Answer from the drawing. Dimensions are ordinates in mm from the lowest x, y and z of the part. Give positions to 0.01 mm unless a question says otherwise; leave off trailing zeros. Loops run counter-clockwise (first coordinate to the right, second up) from the corner with the lowest first, then second, coordinate; pieces in that order, holes last. Notation, with made-up numbers: (63.25, -17) -> (91.25, -17) arc R20 cw to (91.25, 15) -> close; hole circle Ø3 at (21.5, -24). An arc over 180 degrees is marked (long way). Write each question's results on one line, items separated by ' | '. Start each with the question number.
Item 1: Section A-A on z = 472 is taken. Write down the section's boundary in (x, y), and give its area (3 significant figures).
Item 2: Section B-B on x = 26.5 is taken. Write down the section's boundary in (y, z), and give its area (3 significant figures).
Item 3: Section C-C on y = 9 is taken. Write down the section's boundary in (x, z), and give its area (3 significant figures).
Item 4: Each of these flat-tipped pins is pushed along its axis until it touches: P1, Ø10, axis at x = 24, y = 36.5, coming from the -Z side; P2, Ø6, axis at x = 26, y = 35, coming from the +Z side. Where does it stop, or does it pass through?
Item 5: Find the intervals of material crossed by line 1 (X direction, y = 41.5, z = 467.5); line 2 (Z direction, x = 36.5, y = 62), in increasing order.
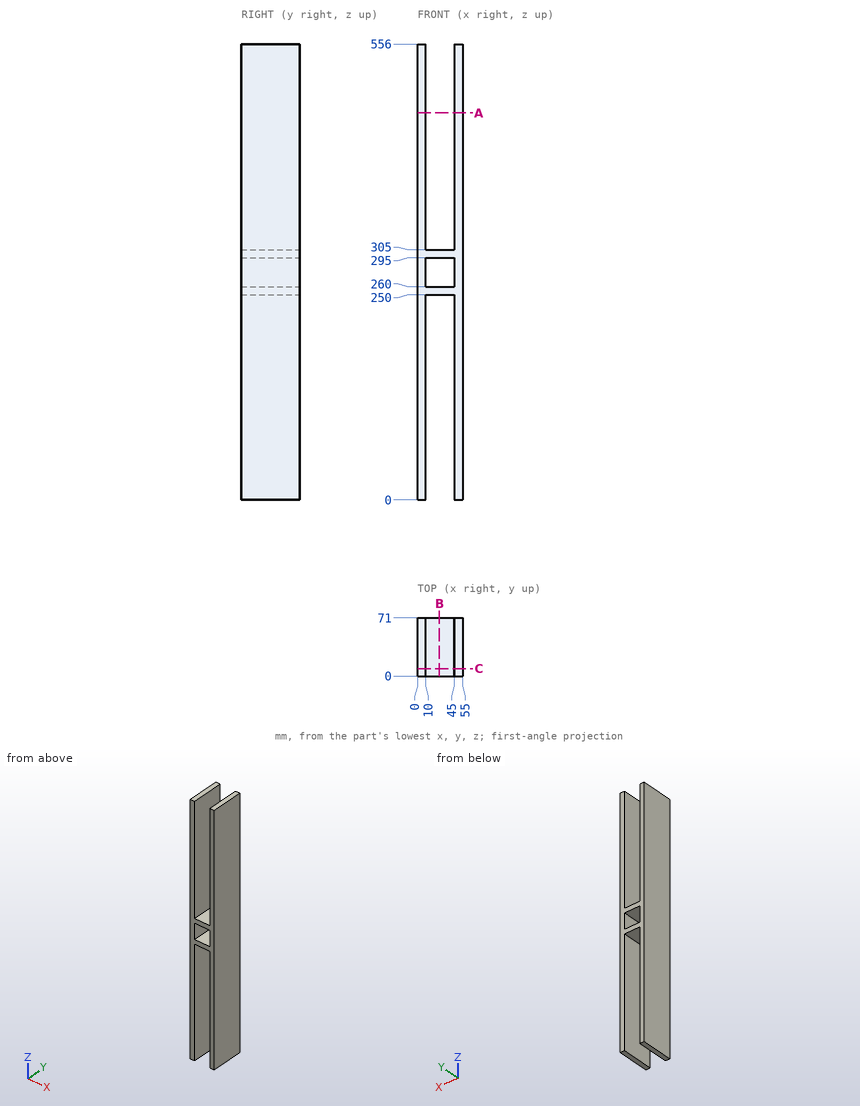
Findings:
1) outline: (0, 0) -> (10, 0) -> (10, 71) -> (0, 71) -> close; (45, 0) -> (55, 0) -> (55, 71) -> (45, 71) -> close | area: 1,420 mm2
2) outline: (0, 250) -> (71, 250) -> (71, 260) -> (0, 260) -> close; (0, 295) -> (71, 295) -> (71, 305) -> (0, 305) -> close | area: 1,420 mm2
3) outline: (0, 0) -> (10, 0) -> (10, 250) -> (45, 250) -> (45, 0) -> (55, 0) -> (55, 556) -> (45, 556) -> (45, 305) -> (10, 305) -> (10, 556) -> (0, 556) -> close; hole (10, 260) -> (45, 260) -> (45, 295) -> (10, 295) -> close | area: 11,800 mm2
4) P1: z = 250 | P2: z = 305
5) line 1: 0 to 10, 45 to 55 | line 2: 250 to 260, 295 to 305
